Design review of the part built by this model. Coordinates are the model's own, in mm. Face numbers are marked on the shaded views. A direction names the side the tool comes from. Coordinates: 2 decimals unless noted, no trailing zeros. Write each loop counter-clockwise with the first axis right and the second up, starting at its lowest first coordinate (ties: lowest second). Pieces come first, ordered by that corner, then holes. Notation, with made-up numbers: (-26, 0.25) -> (8, 0.25) arc R27 ccw to (8, 30.25) -> close; hole circle Ø9 at (40, -34.75). An arc over 180 degrees is marked (long way). One line per question, with ' | ' between items. Start each with the question number.
Q1. Add section B-B on x = -44. State the section outline as (y, z) points.
Q2. Add section C-C on y = 83. State the section outline as (x, z) points.
Q3. For P1, Ø1, axis at x = -42, z = 14.5, coming from the +Y side; P2, Ø2, axis at x = -37, y = 32.5, coming from the +Z side; P3, Ø8, axis at y = -11.5, z = -8, coming from the -X side; P4, Ø19, axis at x = 30, y = 25, coming from the -Z side, all flat-tipped, find the tip position at first contact; note any pin that passes through.
Q4. Add section D-D on z = -35. State the section outline as (x, y) points.
Q5. For the marked faces 1, 2 and 3, list the 3-axis set-ups (+Z, -Z, +X, -X, +Y, -Y) from which the entire face can be reached by the end or side of a thin tool; tool diameter is ignored.
Q6. Wall thickness on probe 1 along X at (y, z) = (121, 24); probe 2 along Y at (x, z) = (44, 24); probe 3 along Z at (x, y) = (-8, 66.5): over which ranges is each line inside the solid? List them lowest first.
Q7. Add section A-A on y = 25. State the section outline as (x, z) points, and give its area (3 significant figures).
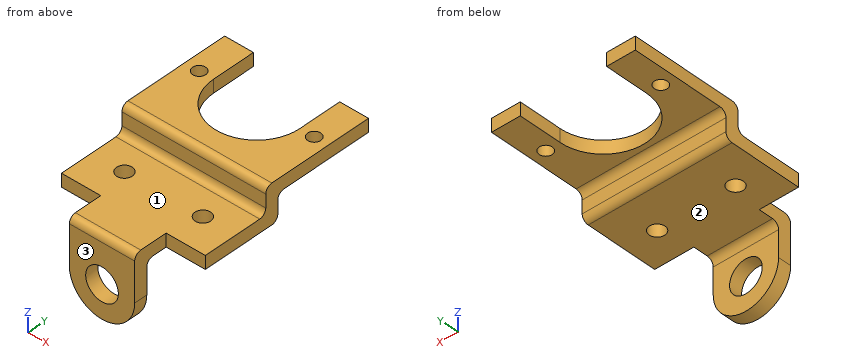
from build123d import *

# Parameters (mm, degrees)
SKETCH_1_R           = 6
EXTRUDE_1_DEPTH      = 10
SKETCH_2_W           = 50
SKETCH_2_H           = 10
EXTRUDE_2_DEPTH      = 60
SKETCH_3_R           = 12.5
CUT_EXTRUDE_1_DEPTH  = 10
FILLET_1_R           = 5
EXTRUDE_3_DEPTH      = 10
EXTRUDE_3_DEPTH_BACK = 10
SKETCH_5_W           = 110
SKETCH_5_H           = 10
SKETCH_6_R           = 5
EXTRUDE_4_DEPTH      = 10
FILLET_2_R           = 5


with BuildPart() as part:
    # 草图1 → 凸台-拉伸1 (new body)
    with BuildSketch(Plane.XY):
        Polygon((-55, 50), (55, 50), (55, 0), (50, 0), (25, 0), (25, -16), (-25, -16), (-25, 0), (-55, 0), align=None)
        with Locations((-30, 25)):
            Circle(SKETCH_1_R, mode=Mode.SUBTRACT)
        with Locations((30, 25)):
            Circle(SKETCH_1_R, mode=Mode.SUBTRACT)
    extrude(amount=EXTRUDE_1_DEPTH)

    # 草图2 → 凸台-拉伸2 (add)
    with BuildSketch(Plane.XY.offset(10)):
        with Locations((0, -21)):
            Rectangle(SKETCH_2_W, SKETCH_2_H)
    extrude(amount=-EXTRUDE_2_DEPTH)

    # 草图3 → 切除-拉伸1 (cut)
    with BuildSketch(Plane(origin=(0, -16, 0), x_dir=(1, 0, 0), z_dir=(0, 1, 0))):
        with Locations(Location((0, 25, 0), (0, 0, 180))):
            Circle(SKETCH_3_R)
        with BuildLine():
            Line((-25, 25), (-25, 57.057636161))
            Line((-25, 57.057636161), (25, 57.057636161))
            Line((25, 57.057636161), (25, 25))
            ThreePointArc((25, 25), (0, 50), (-25, 25))
        make_face()
    extrude(amount=-CUT_EXTRUDE_1_DEPTH, mode=Mode.SUBTRACT)

    # 圆角1
    fillet_1_edges = [part.edges().sort_by_distance(p)[0] for p in [
        (0, -16, 0),
        (0, -26, 10),
    ]]
    fillet(fillet_1_edges, radius=FILLET_1_R)

    # 草图5 → 凸台-拉伸3 (add, two sides: drawn at the far end of the back side and taken through both)
    with BuildSketch(Plane.XY.offset(10).offset(-EXTRUDE_3_DEPTH_BACK)):
        with Locations((0, 55)):
            Rectangle(SKETCH_5_W, SKETCH_5_H)
    extrude(amount=EXTRUDE_3_DEPTH + EXTRUDE_3_DEPTH_BACK)

    # 草图6 → 凸台-拉伸4 (add)
    with BuildSketch(Plane.XY.offset(20)):
        with BuildLine():
            Line((-55, 60), (-55, 135))
            Line((-55, 135), (-33, 135))
            Line((-33, 135), (-33, 102))
            ThreePointArc((-33, 102), (0, 69), (33, 102))
            Line((33, 102), (33, 135))
            Line((33, 135), (55, 135))
            Line((55, 135), (55, 60))
            Line((55, 60), (55, 50))
            Line((55, 50), (-55, 50))
            Line((-55, 50), (-55, 60))
        make_face()
        with Locations((44, 102)):
            Circle(SKETCH_6_R, mode=Mode.SUBTRACT)
        with Locations((-44, 102)):
            Circle(SKETCH_6_R, mode=Mode.SUBTRACT)
    extrude(amount=EXTRUDE_4_DEPTH)

    # 圆角2
    fillet_2_edges = [part.edges().sort_by_distance(p)[0] for p in [
        (0, 50, 10),
        (0, 50, 30),
        (0, 60, 20),
        (0, 60, 0),
    ]]
    fillet(fillet_2_edges, radius=FILLET_2_R)


solid = part.part
Output values:
1) outline: (0, 0) -> (55, 0) arc R5 ccw to (60, 5) -> (60, 15) arc R5 cw to (65, 20) -> (97, 20) -> (97, 30) -> (55, 30) arc R5 ccw to (50, 25) -> (50, 15) arc R5 cw to (45, 10) -> (0, 10) -> close; (107, 20) -> (135, 20) -> (135, 30) -> (107, 30) -> close
2) outline: (-55, 20) -> (-26.98, 20) -> (-26.98, 30) -> (-55, 30) -> close; (26.98, 20) -> (55, 20) -> (55, 30) -> (26.98, 30) -> close
3) P1: stops at y = 60 | P2: stops at z = 10 | P3: passes through | P4: stops at z = 0
4) outline: (-22.91, -26) -> (-7.5, -26) -> (-7.5, -16) -> (-22.91, -16) -> close; (7.5, -26) -> (22.91, -26) -> (22.91, -16) -> (7.5, -16) -> close
5) face 1: +Z, +X, -X, -Y | face 2: -Z, +X, -X, +Y | face 3: +Z, -Z, +X, -X, -Y
6) probe 1: x = -55 to -33, 33 to 55 | probe 2: y = 50 to 97, 107 to 135 | probe 3: z = 20 to 30
7) outline: (-55, 0) -> (-36, 0) -> (-36, 10) -> (-55, 10) -> close; (-24, 0) -> (24, 0) -> (24, 10) -> (-24, 10) -> close; (36, 0) -> (55, 0) -> (55, 10) -> (36, 10) -> close | area: 860 mm2
